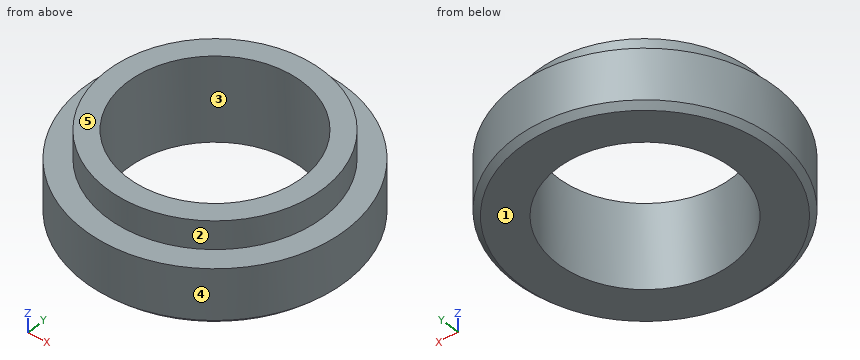
```python
from build123d import *

# Parameters (mm, degrees)
SKETCH1_R             = 19
SKETCH1_R_2           = 7.5
BOSS_EXTRUDE1_DEPTH   = 10
SKETCH2_R             = 23
SKETCH2_R_2           = 7.5
BOSS_EXTRUDE2_DEPTH   = 10
SKETCH3_R             = 19
SKETCH3_R_2           = 7.5
BOSS_EXTRUDE3_DEPTH   = 5
G1_TAPPED_HOLE1_D     = 30.75
G1_TAPPED_HOLE1_DEPTH = 73.43
G1_TAPPED_HOLE1_TIP   = 9.238232018
SKETCH6_R             = 28.473904373
CUT_EXTRUDE1_DEPTH    = 10
CHAMFER2_SIZE         = 1


with BuildPart() as part:
    # Sketch1 → Boss-Extrude1 (new body)
    with BuildSketch(Plane.XY):
        Circle(SKETCH1_R)
        Circle(SKETCH1_R_2, mode=Mode.SUBTRACT)
    extrude(amount=BOSS_EXTRUDE1_DEPTH)

    # Sketch2 → Boss-Extrude2 (add)
    with BuildSketch(Plane.XY.offset(10)):
        Circle(SKETCH2_R)
        Circle(SKETCH2_R_2, mode=Mode.SUBTRACT)
    extrude(amount=BOSS_EXTRUDE2_DEPTH)

    # Sketch3 → Boss-Extrude3 (add)
    with BuildSketch(Plane.XY.offset(20)):
        Circle(SKETCH3_R)
        Circle(SKETCH3_R_2, mode=Mode.SUBTRACT)
    extrude(amount=BOSS_EXTRUDE3_DEPTH)

    # G1 Tapped Hole1
    with Locations(Plane.XY.offset(25)):
        with Locations((0, 0)):
            Hole(G1_TAPPED_HOLE1_D / 2, depth=G1_TAPPED_HOLE1_DEPTH)
            with Locations((0, 0, -(G1_TAPPED_HOLE1_DEPTH + G1_TAPPED_HOLE1_TIP / 2))):  # 118° drill point
                Cone(0, G1_TAPPED_HOLE1_D / 2, G1_TAPPED_HOLE1_TIP, mode=Mode.SUBTRACT)

    # Sketch6 → Cut-Extrude1 (cut)
    with BuildSketch(Plane.XY):
        Circle(SKETCH6_R)
    extrude(amount=CUT_EXTRUDE1_DEPTH, mode=Mode.SUBTRACT)

    # Chamfer2
    chamfer2_edges = [part.edges().sort_by_distance(p)[0] for p in [
        (-23, 0, 10),
    ]]
    chamfer(chamfer2_edges, length=CHAMFER2_SIZE)


solid = part.part
```
Can you work these out from the model? Positions are in its coordinate system, mm. Face numbers are marked on the shaded views. A direction names the side the tool comes from. Give positions to 0.01 mm unless a question says otherwise; leave off trailing zeros. Order: outer loops, then holes, each group sorted by start corner. A loop starts at its lowest first (then second) coordinate and runs counter-clockwise, first axis right, second up. Notation, with made-up numbers: M 48,31.25 L 102,31.25 A17 ccw 102,38.25 Z; hole C 33.5,53.25 d6. An arc over 180 degrees is marked long. Write item = value, one per line. Start each with the question number.
Q1. Will these pins go through, and if not, where does the flat tip stop? pin 1 Ø1 at (x, z) = (3.5, 13) entering from +Y; pin 2 Ø1 at (x, z) = (6.5, 23) entering from -Y; pin 3 Ø8 at (y, z) = (-10, 18) entering from -X.
Q2. I need wall thicknesses on probe 1 along Y at (x, z) = (0, 15) (3 decimals); probe 2 along Y at (x, z) = (0, 21.75) (3 decimals); probe 3 along X at (y, z) = (-8, 12.5). Which ranges of each line are inside material? Lowest first, please. Write a range as [from, to].
Q3. We'd pull the mould along Y, two halves only. Please class the marked faces 3, 4 and 5: pulls with the +Y half, pulls with the -Y half, needs draft (parallel to the pull), parting line crosses it, or undercut.
Q4. Suppose I cut it at D-D (z = 20.75). Write out the boundary of the cut face in (x, y) (3 decimals), plus the area to 3 significant figures.
Q5. Suppose I cut it at A-A (y = 0). Write out the boundary of the cut face in (x, z) (3 decimals).
Q6. Suppose I cut it at C-C (z = 15.5). Write out the boundary of the cut face in (x, y) (3 decimals).
Q7. For the marked faces 1 and 2, which set-ups out of +Z, -Z, +X, -X, +Y, -Y let a thin tool reach every point of the face, with its end or its side?
Check result:
q1.pin_1 = 22.8
q1.pin_2 = -18.03
q1.pin_3 = -22.2
q2.probe_1 = [-23, -15.375], [15.375, 23]
q2.probe_2 = [-19, -15.375], [15.375, 19]
q2.probe_3 = [-21.56, -13.13], [13.13, 21.56]
q3.face_3 = undercut
q3.face_4 = parting line crosses it
q3.face_5 = needs draft
q4.outline = C 0,0 d38; hole C 0,0 d30.75
q4.area = 391 mm2
q5.outline = M -23,11 L -22,10 L -15.375,10 L -15.375,25 L -19,25 L -19,20 L -23,20 Z; M 15.375,10 L 22,10 L 23,11 L 23,20 L 19,20 L 19,25 L 15.375,25 Z
q6.outline = C 0,0 d46; hole C 0,0 d30.75
q7.face_1 = -Z, +X, -X, +Y, -Y
q7.face_2 = +Z
